Work out the finished part from the listing and answer in its coordinate system (mm). A direction names the side the tool comes from. Give positions to 0.01 mm unless a question says otherwise; leave off trailing zeros. Write each loop counter-clockwise with the first axis right and the second up, starting at its lowest first coordinate (ties: lowest second). Pieces come first, ordered by that corner, then holes. Notation, with made-up numbers: (-8, 59) - (20, 59) arc R34 cw to (20, 97) - close; hole circle Ø5 at (54, 80.5). An arc over 180 degrees is marked (long way). Write each question's results on one line, items separated by ' | '. Start each with the question number.
from build123d import *

# Parameters (mm, degrees)
EXTRUDE_1_DEPTH        = 10
HOLE_WIZARD_M6_2_D     = 5
HOLE_WIZARD_M6_2_DEPTH = 20
HOLE_WIZARD_M6_2_TIP   = 1.502151548
HOLE_WIZARD_M6_1_D     = 5
HOLE_WIZARD_M6_1_DEPTH = 20
HOLE_WIZARD_M6_1_TIP   = 1.502151548


with BuildPart() as part:
    # 草图1 → 凸台-拉伸1 (new body)
    with BuildSketch(Plane.XY):
        Polygon((-30, 30), (-30, -30), (30, -30), align=None)
    extrude(amount=EXTRUDE_1_DEPTH)

    # M6 螺纹孔2
    with Locations(Plane(origin=(0, -30, 0), x_dir=(-1, 0, 0), z_dir=(0, -1, 0))):
        with Locations((10, -5), (-20, -5)):
            Hole(HOLE_WIZARD_M6_2_D / 2, depth=HOLE_WIZARD_M6_2_DEPTH)
            with Locations((0, 0, -(HOLE_WIZARD_M6_2_DEPTH + HOLE_WIZARD_M6_2_TIP / 2))):  # 118° drill point
                Cone(0, HOLE_WIZARD_M6_2_D / 2, HOLE_WIZARD_M6_2_TIP, mode=Mode.SUBTRACT)

    # M6 螺纹孔1
    with Locations(Plane.ZY.offset(30)):
        with Locations((5, 20), (5, -10)):
            Hole(HOLE_WIZARD_M6_1_D / 2, depth=HOLE_WIZARD_M6_1_DEPTH)
            with Locations((0, 0, -(HOLE_WIZARD_M6_1_DEPTH + HOLE_WIZARD_M6_1_TIP / 2))):  # 118° drill point
                Cone(0, HOLE_WIZARD_M6_1_D / 2, HOLE_WIZARD_M6_1_TIP, mode=Mode.SUBTRACT)


solid = part.part
Q1. Consider L1, parallel to Y at x = -25, z = 3; L2, parallel to Y at x = -18, z = 5; L3, parallel to Z at x = 20, y = -24. Determine where each line is inside the solid, lowest interval first.
Q2. The mould has two halves that part along Z. Classify faces 4 (the flat face through (-30, 0, 5)), 5 (the flat face through (-14, -13, 0)), 6 (the flat face through (-14, -13, 10)), 7 (the conical face through (-8.617, -9.329, 4.97)): pulls with the +Z half, pulls with the -Z half, needs draft (parallel to the pull), parting line crosses it, or undercut.
Q3. A tool of negligible diameter and unlimited length cuts with its end or side. For faces 1 (the cylindrical face through (-7.615, -19.86, 4.249)), 2 (the cylindrical face through (17.5, -25, 4.9)), 3 (the cylindrical face through (-19.86, -7.89, 3.66)), from which of +Z, -Z, +X, -X, +Y, -Y can it reach the whole face along a straight path? Write none if from no direction.
Q4. A cutting plane is placed at D-D, the plane x = -14. Write down the section's boundary in (y, z), and give its area (3 significant figures).
Q5. A cutting plane is placed at A-A, the plane z = 5. Write down the section's boundary in (x, y).
Q6. A cutting plane is placed at B-B, the plane x = 20. Write down the section's boundary in (y, z).
Q7. Given pin 1 (12 mm diameter, centred on x = -13.5, y = 23, fed in from -Z); pin 2 (4.5 mm diameter, centred on y = -10, z = 5, fed in from +X); pin 3 (3 mm diameter, centred on x = -10, z = 5, fed in from +Y); pin 4 (4 mm diameter, centred on x = -12, z = 5.5, fed in from -Y), each flat-ended and moving along its own axis, determine where each tip first touches the part or whether it passes through.
Result:
1) L1: y = -30 to -11.5, -8.5 to 18.5, 21.5 to 25 | L2: y = -30 to -12.5, -7.5 to 17.5 | L3: z = 0 to 2.5, 7.5 to 10
2) face 4: needs draft | face 5: pulls with the -Z half | face 6: pulls with the +Z half | face 7: undercut
3) face 1: -Y | face 2: +Y, -Y | face 3: -X
4) outline: (-30, 0) - (14, 0) - (14, 10) - (-30, 10) - close; hole circle Ø5 at (-10, 5) | area: 420 mm2
5) outline: (-30, -30) - (-12.5, -30) - (-12.5, -12.5) - (-30, -12.5) - close; (-30, -7.5) - (-10, -7.5) - (-9.06, -9.06) - (-7.5, -10) - (-7.5, -30) - (17.5, -30) - (17.5, -17.5) - (-17.5, 17.5) - (-30, 17.5) - close; (-30, 22.5) - (-22.5, 22.5) - (-30, 30) - close; (22.5, -30) - (30, -30) - (22.5, -22.5) - close
6) outline: (-30, 0) - (-20, 0) - (-20, 2.5) - (-30, 2.5) - close; (-30, 7.5) - (-20, 7.5) - (-20, 10) - (-30, 10) - close
7) pin 1: passes through | pin 2: stops at x = 12.25 | pin 3: stops at y = 11.5 | pin 4: stops at y = -30
